from build123d import *

# Parameters (mm, degrees)
BASE_BLOCK_DEPTH               = 60
CLEVIS_LUG_DEPTH               = 20
LUG_EXTENSION_DEPTH            = 20
PIN_HOLE_SKETCH_30_R           = 15
CLEVIS_PIN_HOLE_30_DEPTH       = 215
UPRIGHT_WEB_DEPTH              = 20
FLANGE_PLATE_DEPTH             = 20
WEB_FLANGE_FILLET_R20_A_R      = 20
WEB_FLANGE_FILLET_R20_B_R      = 20
WEB_BASE_FILLET_R20_A_R        = 20
WEB_BASE_FILLET_R20_B_R        = 20
HUB_BOSS_DEPTH                 = 35
HUB_WEB_FILLET_R20_A_R         = 20
HUB_WEB_FILLET_R20_B_R         = 20
MOUNTING_BOSSES_SKETCH_2X_40_R = 20
MOUNTING_BOSSES_2X_40_DEPTH    = 30
MOUNTING_BOSS_FILLET_R5_A_R    = 5
MOUNTING_BOSS_FILLET_R5_B_R    = 5
HUB_BORE_SKETCH_50_R           = 25
HUB_BORE_50_DEPTH              = 82
MOUNTING_HOLES_SKETCH_2X_20_R  = 10
MOUNTING_HOLES_2X_20_DEPTH     = 82


with BuildPart() as part:
    # Base Profile Sketch → Base Block (new body)
    with BuildSketch(Plane.XY):
        Polygon((60, 0), (80, 0), (80, 60), (-80, 60), (-80, 0), (-60, 0), (-60, 40), (60, 40), align=None)
    extrude(amount=BASE_BLOCK_DEPTH)

    # Clevis Lug Sketch → Clevis Lug (add)
    with BuildSketch(Plane(origin=(0, 60, 0), x_dir=(1, 0, 0), z_dir=(0, 1, 0))):
        Polygon((0, -135), (33, -135), (33, -60), (-33, -60), (-33, -135), align=None)
    extrude(amount=-CLEVIS_LUG_DEPTH)

    # Lug Extension Sketch → Lug Extension (add)
    with BuildSketch(Plane.XY.offset(135)):
        with BuildLine():
            Line((33, -17), (33, 40))
            Line((33, 40), (-33, 40))
            Line((-33, 40), (-33, -17))
            ThreePointArc((-33, -17), (0, -50), (33, -17))
        make_face()
    extrude(amount=-LUG_EXTENSION_DEPTH)

    # Pin Hole Sketch Ø30 → Clevis Pin Hole Ø30 (cut)
    with BuildSketch(Plane.XY.offset(135)):
        with Locations((0, -17)):
            Circle(PIN_HOLE_SKETCH_30_R)
    extrude(amount=-CLEVIS_PIN_HOLE_30_DEPTH, mode=Mode.SUBTRACT)

    # Upright Web Sketch → Upright Web (add)
    with BuildSketch(Plane(origin=(0, 0, 0), x_dir=(-1, 0, 0), z_dir=(0, 0, -1))):
        Polygon((0, 60), (45, 60), (45, 160), (-45, 160), (-45, 60), align=None)
    extrude(amount=-UPRIGHT_WEB_DEPTH)

    # Flange Plate Sketch → Flange Plate (add)
    with BuildSketch(Plane.XY.offset(20)):
        with BuildLine():
            Line((0, 260), (45, 260))
            Line((45, 260), (109.504258609, 238.45468447))
            ThreePointArc((109.504258609, 238.45468447), (130, 210), (109.504258609, 181.54531553))
            Line((109.504258609, 181.54531553), (45, 160))
            Line((45, 160), (-45, 160))
            Line((-45, 160), (-109.504258609, 181.54531553))
            ThreePointArc((-109.504258609, 181.54531553), (-129.973433228, 208.737739921), (-111.86296755, 237.554854398))
            Line((-111.86296755, 237.554854398), (-45, 260))
            Line((-45, 260), (0, 260))
        make_face()
    extrude(amount=-FLANGE_PLATE_DEPTH)

    # Web-Flange Fillet R20 A
    web_flange_fillet_r20_a_edges = [part.edges().sort_by_distance(p)[0] for p in [
        (-45, 160, 10),
    ]]
    fillet(web_flange_fillet_r20_a_edges, radius=WEB_FLANGE_FILLET_R20_A_R)

    # Web-Flange Fillet R20 B
    web_flange_fillet_r20_b_edges = [part.edges().sort_by_distance(p)[0] for p in [
        (45, 160, 10),
    ]]
    fillet(web_flange_fillet_r20_b_edges, radius=WEB_FLANGE_FILLET_R20_B_R)

    # Web-Base Fillet R20 A
    web_base_fillet_r20_a_edges = [part.edges().sort_by_distance(p)[0] for p in [
        (45, 60, 10),
    ]]
    fillet(web_base_fillet_r20_a_edges, radius=WEB_BASE_FILLET_R20_A_R)

    # Web-Base Fillet R20 B
    web_base_fillet_r20_b_edges = [part.edges().sort_by_distance(p)[0] for p in [
        (-45, 60, 10),
    ]]
    fillet(web_base_fillet_r20_b_edges, radius=WEB_BASE_FILLET_R20_B_R)

    # Hub Sketch → Hub Boss (add, symmetric)
    with BuildSketch(Plane(origin=(0, 210, 0), x_dir=(1, 0, 0), z_dir=(0, 1, 0))):
        with BuildLine():
            Line((-45, -75), (-45, -20))
            Line((-45, -20), (45, -20))
            Line((45, -20), (45, -75))
            ThreePointArc((45, -75), (0, -120), (-45, -75))
        make_face()
    extrude(amount=HUB_BOSS_DEPTH, both=True)

    # Hub-Web Fillet R20 A
    hub_web_fillet_r20_a_edges = [part.edges().sort_by_distance(p)[0] for p in [
        (-45, 210, 20),
    ]]
    fillet(hub_web_fillet_r20_a_edges, radius=HUB_WEB_FILLET_R20_A_R)

    # Hub-Web Fillet R20 B
    hub_web_fillet_r20_b_edges = [part.edges().sort_by_distance(p)[0] for p in [
        (45, 210, 20),
    ]]
    fillet(hub_web_fillet_r20_b_edges, radius=HUB_WEB_FILLET_R20_B_R)

    # Mounting Bosses Sketch 2xØ40 → Mounting Bosses 2xØ40 (add)
    with BuildSketch(Plane.XY.offset(20)):
        with Locations(Location((100, 210, 0), (0, 0, 180))):
            Circle(MOUNTING_BOSSES_SKETCH_2X_40_R)
        with Locations(Location((-100, 210, 0), (0, 0, 180))):
            Circle(MOUNTING_BOSSES_SKETCH_2X_40_R)
    extrude(amount=MOUNTING_BOSSES_2X_40_DEPTH)

    # Mounting Boss Fillet R5 A
    mounting_boss_fillet_r5_a_edges = [part.edges().sort_by_distance(p)[0] for p in [
        (120, 210, 20),
    ]]
    fillet(mounting_boss_fillet_r5_a_edges, radius=MOUNTING_BOSS_FILLET_R5_A_R)

    # Mounting Boss Fillet R5 B
    mounting_boss_fillet_r5_b_edges = [part.edges().sort_by_distance(p)[0] for p in [
        (-80, 210, 20),
    ]]
    fillet(mounting_boss_fillet_r5_b_edges, radius=MOUNTING_BOSS_FILLET_R5_B_R)

    # Hub Bore Sketch Ø50 → Hub Bore Ø50 (cut)
    with BuildSketch(Plane(origin=(0, 245, 0), x_dir=(1, 0, 0), z_dir=(0, 1, 0))):
        with Locations(Location((0, -75, 0), (0, 0, 270))):
            Circle(HUB_BORE_SKETCH_50_R)
    extrude(amount=-HUB_BORE_50_DEPTH, mode=Mode.SUBTRACT)

    # Mounting Holes Sketch 2xØ20 → Mounting Holes 2xØ20 (cut)
    with BuildSketch(Plane.XY.offset(50)):
        with Locations((100, 210)):
            Circle(MOUNTING_HOLES_SKETCH_2X_20_R)
        with Locations((-100, 210)):
            Circle(MOUNTING_HOLES_SKETCH_2X_20_R)
    extrude(amount=-MOUNTING_HOLES_2X_20_DEPTH, mode=Mode.SUBTRACT)


solid = part.part
Input: part model. Units: mm. Frame: model coordinates. A direction names the side the tool comes from. Coordinates: 2 decimals unless noted, no trailing zeros. Loops run counter-clockwise (first coordinate to the right, second up) from the corner with the lowest first, then second, coordinate; pieces in that order, holes last. Notation, with made-up numbers: (85.5, 29) -> (138.5, 29) arc R24 cw to (138.5, 44) -> close; hole circle Ø4 at (6.5, -1.5). An arc over 180 degrees is marked (long way). One line per item, written item: value.
(1) Set-up query: faces 1 (the face through (-85.26, 196.48, 37.33)), 2 (the face through (-60, 20, 30)), 3 (the face through (48.67, 157.14, 10.14)), 4 (the face through (33, 38, 123)). Return all of +Z, -Z, +X, -X, +Y, -Y with unobstructed straight access to the full face (end or side cutting, diameter ignored); none if empty.
Answer below:
face 1: +Z
face 2: +Z, -Z, -Y
face 3: +Z, -Z, +X
face 4: +Z, +X, -Y
(2) Cut plane B-B (x = 0). Output: boundary loops of the cut face in (y, z).
Answer below:
outline: (-50, 115) -> (-32, 115) -> (-32, 135) -> (-50, 135) -> close; (-2, 115) -> (40, 115) -> (40, 0) -> (260, 0) -> (260, 20) -> (245, 20) -> (245, 50) -> (175, 50) -> (175, 20) -> (60, 20) -> (60, 135) -> (-2, 135) -> close; (175, 100) -> (245, 100) -> (245, 120) -> (175, 120) -> close
(3) Pin query (flat end, axial travel): pin 1 Ø3 at (x, y) = (27.5, -7) entering from -Z; pin 2 Ø16 at (x, z) = (-65, 37.5) entering from -Y; pin 3 Ø12 at (x, z) = (-32, 83) entering from -Y. Return the tip coordinate at first contact, or that it passes through.
Answer below:
pin 1: stops at z = 115
pin 2: stops at y = 0
pin 3: stops at y = 40
(4) Draft query along Y for faces 5 (the face through (-1, 40, 44)), 6 (the face through (-45, 210, 58)), 7 (the face through (-107.37, 216.76, 25.35)), 8 (the face through (-1.953, -2.128, 125.14)). Return one class per face: pulls with the +Y half, pulls with the -Y half, needs draft (parallel to the pull), parting line crosses it, or undercut.
Answer below:
face 5: pulls with the -Y half
face 6: needs draft
face 7: undercut
face 8: undercut
(5) Cut plane A-A (y = 210). Give the number of separate pieces and of enclosed holes in the cut face, then the cut area to 3 significant figures.
Answer below:
separate pieces: 3
enclosed holes: 1
area: 12,000 mm2
(6) Ray query, line 1 along Y through (x, z) = (0, 126); line 2 along Y through (x, z) = (14, 20.5); line 3 along X through (y, z) = (19, 53). Return the intervals inside material, ascending.
Answer below:
line 1: y = -50 to -32, -2 to 60
line 2: y = 40 to 60, 175 to 245
line 3: x = -80 to -60, 60 to 80
(7) Cut plane C-C (y = 9.5). Output: boundary loops of the cut face in (x, z), then the cut area to 3 significant figures.
Answer below:
outline: (-80, 0) -> (-60, 0) -> (-60, 60) -> (-80, 60) -> close; (-33, 115) -> (33, 115) -> (33, 135) -> (-33, 135) -> close; (60, 0) -> (80, 0) -> (80, 60) -> (60, 60) -> close
area: 3,720 mm2
(8) Cut plane D-D (z = 29). Output: boundary loops of the cut face in (x, y).
Answer below:
outline: circle Ø40 at (-100, 210); (-80, 0) -> (-60, 0) -> (-60, 40) -> (60, 40) -> (60, 0) -> (80, 0) -> (80, 60) -> (-80, 60) -> close; (-48.3, 175) -> (48.3, 175) -> (48.3, 245) -> (-48.3, 245) -> close; circle Ø40 at (100, 210); hole circle Ø20 at (-100, 210); hole circle Ø20 at (100, 210)
